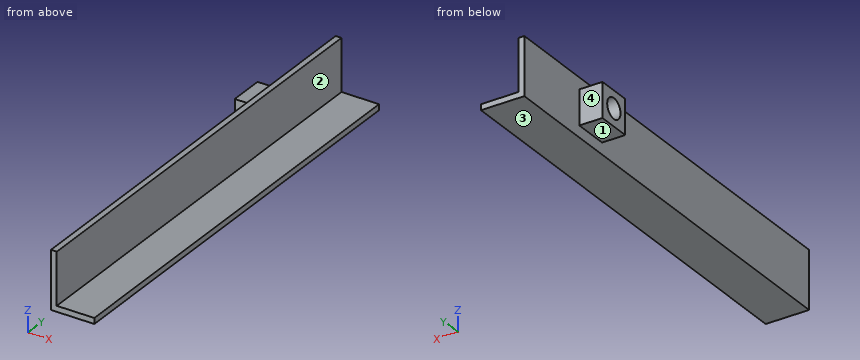
from build123d import *

# Parameters (mm, degrees)
SKETCH1_W           = 15
SKETCH1_H           = 70
BOSS_EXTRUDE1_DEPTH = 20
SKETCH2_W           = 13
SKETCH2_H           = 18
CUT_EXTRUDE1_DEPTH  = 154
BOSS_EXTRUDE2_DEPTH = 80
SKETCH4_W           = 12
SKETCH4_H           = 12
SKETCH4_R           = 3.5
BOSS_EXTRUDE4_DEPTH = 10


with BuildPart() as part:
    # Sketch1 → Boss-Extrude1 (new body)
    with BuildSketch(Plane.XY):
        with Locations((100, 0)):
            Rectangle(SKETCH1_W, SKETCH1_H)
    extrude(amount=BOSS_EXTRUDE1_DEPTH)

    # Sketch2 → Cut-Extrude1 (cut)
    with BuildSketch(Plane(origin=(0, -35, 0), x_dir=(-1, 0, 0), z_dir=(0, -1, 0))):
        with Locations((-101, -11)):
            Rectangle(SKETCH2_W, SKETCH2_H)
    extrude(amount=-CUT_EXTRUDE1_DEPTH, mode=Mode.SUBTRACT)

    # Sketch3 → Boss-Extrude2 (add)
    with BuildSketch(Plane.XZ.offset(35)):
        Polygon((107.5, 0), (107.5, 2), (94.5, 2), (94.5, 20), (92.5, 20), (92.5, 0), align=None)
    extrude(amount=BOSS_EXTRUDE2_DEPTH)

    # Sketch4 → Boss-Extrude4 (add)
    with BuildSketch(Plane(origin=(94.5, 0, 0), x_dir=(0, 0, -1), z_dir=(1, 0, 0))):
        with Locations((-10, 0)):
            Rectangle(SKETCH4_W, SKETCH4_H)
        with Locations(Location((-10, 0, 0), (0, 0, 90))):
            Circle(SKETCH4_R, mode=Mode.SUBTRACT)
    extrude(amount=-BOSS_EXTRUDE4_DEPTH)


solid = part.part
Could you check a few things on this model? Use its own coordinates, in mm. Face numbers are marked on the shaded views. A direction names the side the tool comes from. Coordinates: 2 decimals unless noted, no trailing zeros. Order: outer loops, then holes, each group sorted by start corner. A loop starts at its lowest first (then second) coordinate and runs counter-clockwise, first axis right, second up. Notation, with made-up numbers: (-35.5, 52) -> (15.5, 52) arc R18 ccw to (15.5, 86) -> close; hole circle Ø10 at (41.25, 19.5). An arc over 180 degrees is marked (long way). One line per item, written item: value. Start each with the question number.
1) Imagine slicing it at A-A on z = 10. List the corners of the cut face in (x, y) for me.
2) Which directions (+Z, -Z, +X, -X, +Y, -Y) give clear straight access to the entire face, cutting with the end or side of a thin tool? Please do the marked faces 1, 2, 3 and 4.
3) Imagine slicing it at B-B on x = 90.5. List the corners of the cut face in (y, z) for me, plus the area to 3 significant figures.
4) I'm going to push flat-ended pins straight in: pin 1 (2 mm diameter, centred on y = -1.5, z = 9, fed in from -X); pin 2 (10 mm diameter, centred on y = -61.5, z = 12.5, fed in from +X); pin 3 (9 mm diameter, centred on y = 0, z = 10, fed in from -X); pin 4 (2.5 mm diameter, centred on x = 88.5, y = 0, fed in from +Z). Where does each tip first touch, or does it pass through?
5) Imagine slicing it at C-C on y = 0. List the corners of the cut face in (x, z) for me.
6) Imagine slicing it at D-D on y = -68.5. List the corners of the cut face in (x, z) for me, plus the area to 3 significant figures.
7) If I drill on L1, parallel to Z at x = 90.5, y = 0; L2, parallel to X at y = -107.5, z = 9.25; L3, parallel to Z at x = 105.5, y = -44, over which ranges is the centre line in solid material (lowest first)? Write a range as [from, to].
Answer list:
1. outline: (84.5, -6) -> (92.5, -6) -> (92.5, -115) -> (94.5, -115) -> (94.5, 35) -> (92.5, 35) -> (92.5, 6) -> (84.5, 6) -> (84.5, 3.5) -> (92.5, 3.5) -> (92.5, -3.5) -> (84.5, -3.5) -> close
2. face 1: -Z, -X, +Y, -Y
2. face 2: +Z, +X, +Y, -Y
2. face 3: -Z, +X, -X, +Y, -Y
2. face 4: +Z, -Z, -X, +Y
3. outline: (-6, 4) -> (6, 4) -> (6, 16) -> (-6, 16) -> close; hole circle Ø7 at (0, 10)
3. area: 106 mm2
4. pin 1: stops at x = 92.5
4. pin 2: stops at x = 94.5
4. pin 3: stops at x = 84.5
4. pin 4: stops at z = 16
5. outline: (84.5, 4) -> (92.5, 4) -> (92.5, 0) -> (107.5, 0) -> (107.5, 2) -> (94.5, 2) -> (94.5, 20) -> (92.5, 20) -> (92.5, 16) -> (84.5, 16) -> (84.5, 13.5) -> (92.5, 13.5) -> (92.5, 6.5) -> (84.5, 6.5) -> close
6. outline: (92.5, 0) -> (107.5, 0) -> (107.5, 2) -> (94.5, 2) -> (94.5, 20) -> (92.5, 20) -> close
6. area: 66.0 mm2
7. L1: z = [4, 6.5], [13.5, 16]
7. L2: x = [92.5, 94.5]
7. L3: z = [0, 2]
